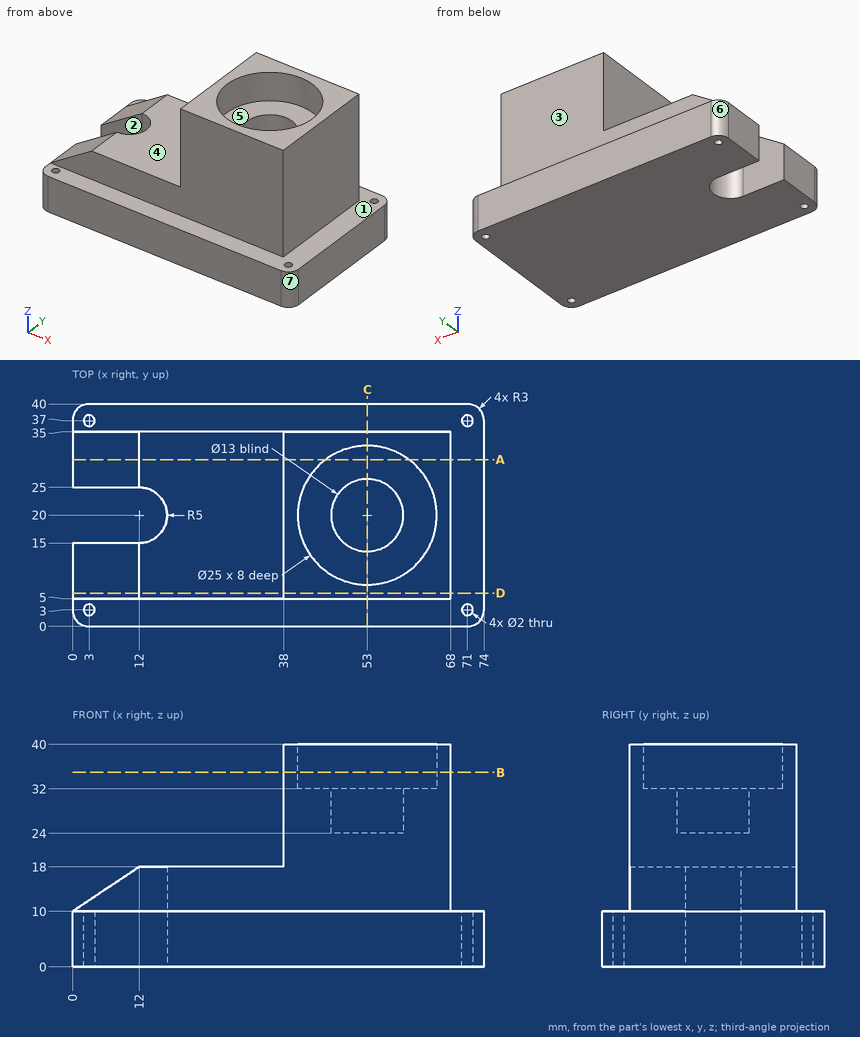
Could you check a few things on this drawing? It's one solid part, dimensions in mm from its lowest x, y, z. A direction names the side the tool comes from. Round coordinates to 2 decimals unless told otherwise and drop trailing zeros. Order: outer loops, then holes, each group sorted by start corner. A loop starts at its lowest first (then second) coordinate and runs counter-clockwise, first axis right, second up. Notation, with made-up numbers: M 88,63 L 112,63 A33 cw 112,100 Z; hole C 85.5,-24 d3. An arc over 180 degrees is marked long. One line per question, with ' | ' between items.
1) Imagine slicing it at D-D, the plane y = 6. Write out the boundary of the cut face in (x, z), plus the area to 3 significant figures.
Checked values:
outline: M 0,0 L 74,0 L 74,10 L 68,10 L 68,40 L 38,40 L 38,18 L 12,18 L 0,10 Z | area: 1,900 mm²
2) On a 3-axis mill with a long thin cutter (end or side, diameter ignored), from which of +Z, -Z, +X, -X, +Y, -Y can I reach the whole of each face in a straight line? I mean the marked faces 1, 2, 3 and 4. Say none if no direction works.
Checked values:
face 1: +Z, +X | face 2: +Z, -Z, -X | face 3: +Z, +X, -X, +Y | face 4: +Z, -X, +Y, -Y
3) We'd pull the mould along X, two halves only. Please class the marked faces 5, 6 and 7: released by +X, released by -X, zero draft, split by the parting line, or undercut.
Checked values:
face 5: undercut | face 6: released by -X | face 7: released by +X
4) Imagine slicing it at B-B, the plane z = 35. Write out the boundary of the cut face in (x, y).
Checked values:
outline: M 38,5 L 68,5 L 68,35 L 38,35 Z; hole C 53,20 d25
5) Imagine slicing it at C-C, the plane x = 53. Write out the boundary of the cut face in (y, z), plus the area to 3 significant figures.
Checked values:
outline: M 0,0 L 40,0 L 40,10 L 35,10 L 35,40 L 32.5,40 L 32.5,32 L 26.5,32 L 26.5,24 L 13.5,24 L 13.5,32 L 7.5,32 L 7.5,40 L 5,40 L 5,10 L 0,10 Z | area: 996 mm²
6) I need wall thicknesses on line 1 (Y direction, x = 3, z = 6); line 2 (Y direction, x = 53, z = 35); line 3 (Y direction, x = 71, z = 7). Which ranges of each line are inside material? Lowest first, please.
Checked values:
line 1: y = 0 to 2, 4 to 15, 25 to 36, 38 to 40 | line 2: y = 5 to 7.5, 32.5 to 35 | line 3: y = 0 to 2, 4 to 36, 38 to 40
7) Imagine slicing it at A-A, the plane y = 30. Write out the boundary of the cut face in (x, z), plus the area to 3 significant figures.
Checked values:
outline: M 0,0 L 74,0 L 74,10 L 68,10 L 68,40 L 60.5,40 L 60.5,32 L 45.5,32 L 45.5,40 L 38,40 L 38,18 L 12,18 L 0,10 Z | area: 1,780 mm²
8) I'm going to push flat-ended pins straight in: pin 1 Ø1.8 at (x, y) = (3, 37) entering from -Z; pin 2 Ø1.5 at (x, z) = (30.5, 16.5) entering from -Y; pin 3 Ø1 at (y, z) = (5.5, 13.5) entering from -X; pin 4 Ø1 at (y, z) = (13, 29) entering from -X. Where does each tip first touch, or does it pass through?
Checked values:
pin 1: passes through | pin 2: stops at y = 5 | pin 3: stops at x = 4.5 | pin 4: stops at x = 38
